For this review, take the finished solid that the model builds, in its own axes (mm). Face numbers are marked on the shaded views. A direction names the side the tool comes from. Coordinates: 2 decimals unless noted, no trailing zeros. Order: outer loops, then holes, each group sorted by start corner. A loop starts at its lowest first (then second) coordinate and runs counter-clockwise, first axis right, second up. Notation, with made-up numbers: (35.25, 66.5) -> (74.25, 66.5) arc R38 ccw to (74.25, 104.5) -> close; hole circle Ø5 at (13, -23.5). An arc over 180 degrees is marked (long way). Write item = value, one per line. Start each with the question number.
1) Draft analysis for pull direction X (two halves, no side actions). For the marked faces 3, 4 and 5, state which applies: +X half, -X half, draft (parallel to the pull), parting line (faces both ways), or undercut.
2) Insertion check: pin 1 Ø2 at (y, z) = (-14.5, -23.5) entering from +X; pin 2 Ø18 at (x, z) = (0, 0) entering from +Y; pin 3 Ø12 at (y, z) = (-10, 10) entering from +X; pin 4 Ø6 at (x, y) = (2, 3) entering from -Z. Each pin has a flat end and moves straight along its axis. Give the tip position at first contact, or say it passes through.
3) Consider section B-B on z = 0. Give the boundary of the cut face in (x, y).
4) Wall thickness on probe 1 along X at (y, z) = (-10.75, 0); probe 2 along X at (y, z) = (6, 0); probe 3 along Z at (x, y) = (-10, 3.5): over which ranges is each line inside the solid? List them lowest first. Write a range as [from, to].
5) Machinability: for the marked faces 1 and 2, which of the approach directions +Z, -Z, +X, -X, +Y, -Y give a long, thin tool a straight path to every point of the face, cutting with its end or side? Answer none if there is none.
6) Consider section D-D on y = -17. Give the boundary of the cut face in (x, z), and give its area (3 significant figures).
7) Consider section C-C on y = 15. Give the boundary of the cut face in (x, z), and give its area (3 significant figures).
8) Consider section A-A on x = 0. Give the boundary of the cut face in (y, z).
from build123d import *


with BuildPart() as part:
    # 草图1 → 旋转1 (revolve)
    with BuildSketch(Plane.XY, mode=Mode.PRIVATE) as revolve_1_sk:
        with BuildLine():
            Line((15, -20), (15, 0))
            Line((15, 0), (18, 0))
            ThreePointArc((18, 0), (19.414213562, 0.585786438), (20, 2))
            Line((20, 2), (20, 20))
            Line((20, 20), (30, 20))
            Line((30, 20), (30, -20))
            Line((30, -20), (15, -20))
        make_face()
    revolve(revolve_1_sk.sketch.rotate(Axis((0, 45.568181818, 0), (0, -1, 0)), 90), axis=Axis((0, 45.568181818, 0), (0, -1, 0)))


solid = part.part
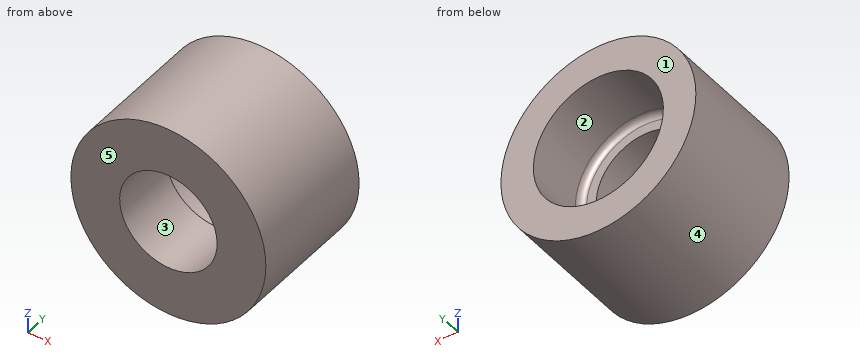
Answer sheet:
q1.face_3 = undercut
q1.face_4 = parting line
q1.face_5 = draft
q2.pin_1 = 19.84
q2.pin_2 = through
q2.pin_3 = 29.73
q2.pin_4 = -30
q3.outline = (-30, -20) -> (-15, -20) -> (-15, 0) -> (-18, 0) arc R2 cw to (-20, 2) -> (-20, 20) -> (-30, 20) -> close; (15, -20) -> (30, -20) -> (30, 20) -> (20, 20) -> (20, 2) arc R2 cw to (18, 0) -> (15, 0) -> close
q4.probe_1 = [-30, -15], [15, 30]
q4.probe_2 = [-30, -20], [20, 30]
q4.probe_3 = [-28.28, -17.32], [17.32, 28.28]
q5.face_1 = +Z, -Z, +X, -X, +Y
q5.face_2 = +Y
q6.outline = circle Ø60 at (0, 0); hole circle Ø30 at (0, 0)
q6.area = 2,120 mm2
q7.outline = circle Ø60 at (0, 0); hole circle Ø40 at (0, 0)
q7.area = 1,570 mm2
q8.outline = (-20, -30) -> (20, -30) -> (20, -20) -> (2, -20) arc R2 cw to (0, -18) -> (0, -15) -> (-20, -15) -> close; (-20, 15) -> (0, 15) -> (0, 18) arc R2 cw to (2, 20) -> (20, 20) -> (20, 30) -> (-20, 30) -> close
